Geometry: final body of the model. Coordinates: model frame, mm. Face numbers are marked on the shaded views. Coordinates: 2 decimals unless noted, no trailing zeros. Write each loop counter-clockwise with the first axis right and the second up, starting at its lowest first coordinate (ties: lowest second). Pieces come first, ordered by that corner, then holes. Notation, with made-up numbers: M -2,89.25 L 4,89.25 A17 ccw 4,115.25 Z; hole C 20.5,-40 d9. An arc over 180 degrees is marked long. Write item = value, one per line. Start each with the question number.
Item 1: Ray query, L1, parallel to Y at x = 0, z = 3.2; L2, parallel to Y at x = 0, z = -3.15; L3, parallel to Y at x = 0, z = 1. Return the intervals inside material, ascending. Write a range as [from, to].
Item 2: Section A-A on x = 0. Output: boundary loops of the cut face in (y, z).
Item 3: First-contact query: pin 1 Ø3 at (x, z) = (7.5, -1) entering from +Y; pin 2 Ø2 at (x, z) = (-9, -1.5) entering from +Y. Flat tips, straight axial feed; report the tip coordinate or a pass-through.
Item 4: Pull-direction query (Y, two-part tool) for the marked faces 1, 2 and 3; classes: +Y half, -Y half, draft (parallel to the pull), parting line (faces both ways), or undercut.
Item 5: Section C-C on y = 26.5. Output: boundary loops of the cut face in (x, z).
from build123d import *

# Parameters (mm, degrees)
EXTRUDE_START   = -2
SKETCH_2_R      = 33.5
SKETCH_2_R_2    = 32.5
EXTRUDE_1_DEPTH = 2


with BuildPart() as part:
    # 草图1 → 旋转1 (revolve)
    with BuildSketch(Plane(origin=(0, 0, 0), x_dir=(0, 0, -1), z_dir=(1, 0, 0)), mode=Mode.PRIVATE) as revolve_1_sk:
        Polygon((-3.5, 25), (-3.5, 27.55), (-3, 27.55), (-3, 29.95), (-3.5, 29.95), (-3.5, 32.5), (3.5, 32.5), (3.5, 29.95), (3, 29.95), (3, 27.55), (3.5, 27.55), (3.5, 25), align=None)
    revolve(revolve_1_sk.sketch.rotate(Axis((0, 0, 0), (0, 0, -1)), 90), axis=Axis((0, 0, 0), (0, 0, -1)))

    # 草图2 → 凸台-拉伸1 (add)
    with BuildSketch(Plane.XY.offset(3.5).offset(EXTRUDE_START)):
        Circle(SKETCH_2_R)
        Circle(SKETCH_2_R_2, mode=Mode.SUBTRACT)
    extrude(amount=EXTRUDE_1_DEPTH)


solid = part.part
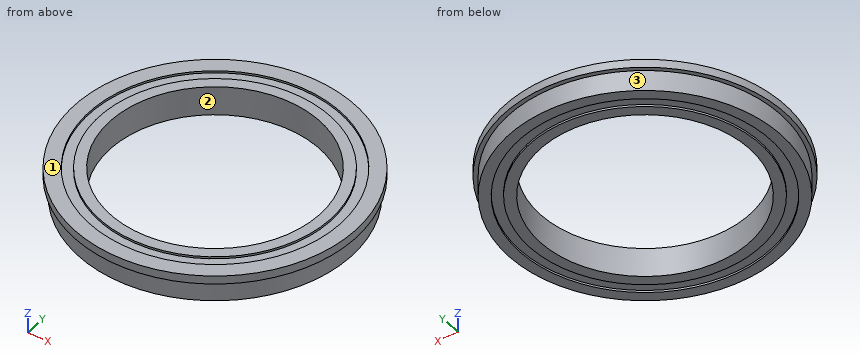
Responses:
q1.L1 = [-33.5, -29.95], [-27.55, -25], [25, 27.55], [29.95, 33.5]
q1.L2 = [-32.5, -29.95], [-27.55, -25], [25, 27.55], [29.95, 32.5]
q1.L3 = [-32.5, -25], [25, 32.5]
q2.outline = M -33.5,1.5 L -32.5,1.5 L -32.5,-3.5 L -29.95,-3.5 L -29.95,-3 L -27.55,-3 L -27.55,-3.5 L -25,-3.5 L -25,3.5 L -27.55,3.5 L -27.55,3 L -29.95,3 L -29.95,3.5 L -33.5,3.5 Z; M 25,-3.5 L 27.55,-3.5 L 27.55,-3 L 29.95,-3 L 29.95,-3.5 L 32.5,-3.5 L 32.5,1.5 L 33.5,1.5 L 33.5,3.5 L 29.95,3.5 L 29.95,3 L 27.55,3 L 27.55,3.5 L 25,3.5 Z
q3.pin_1 = 31.94
q3.pin_2 = 31.5
q4.face_1 = draft
q4.face_2 = undercut
q4.face_3 = parting line
q5.outline = M -20.49,1.5 L -18.81,1.5 L -18.81,-3.5 L -13.96,-3.5 L -13.96,-3 L -7.53,-3 L -7.53,-3.5 L 7.53,-3.5 L 7.53,-3 L 13.96,-3 L 13.96,-3.5 L 18.81,-3.5 L 18.81,1.5 L 20.49,1.5 L 20.49,3.5 L 13.96,3.5 L 13.96,3 L 7.53,3 L 7.53,3.5 L -7.53,3.5 L -7.53,3 L -13.96,3 L -13.96,3.5 L -20.49,3.5 Z
